from build123d import *

# Parameters (mm, degrees)
SKETCH1_R           = 2.9
BOSS_EXTRUDE1_DEPTH = 6.35
BOSS_EXTRUDE2_START = -6.35
SKETCH2_R           = 2.9
SKETCH2_R_2         = 2.6035
BOSS_EXTRUDE2_DEPTH = 6.35


with BuildPart() as part:
    # Sketch1 → Boss-Extrude1 (new body)
    with BuildSketch(Plane(origin=(0, 0, 0), x_dir=(1, 0, 0), z_dir=(0, 1, 0))):
        with BuildLine():
            Line((0, 5.08), (50.8, 5.08))
            ThreePointArc((50.8, 5.08), (55.88, 0), (50.8, -5.08))
            Line((50.8, -5.08), (0, -5.08))
            ThreePointArc((0, -5.08), (-5.08, 0), (0, 5.08))
        make_face()
        with Locations(Location((0, 0, 0), (0, 0, 270))):
            Circle(SKETCH1_R, mode=Mode.SUBTRACT)
        with Locations(Location((50.8, 0, 0), (0, 0, 270))):
            Circle(SKETCH1_R, mode=Mode.SUBTRACT)
    extrude(amount=BOSS_EXTRUDE1_DEPTH)

    # Sketch2 → Boss-Extrude2 (add)
    # profile 1 of 2: a face of its own
    with BuildSketch(Plane(origin=(0, 6.35, 0), x_dir=(1, 0, 0), z_dir=(0, 1, 0)).offset(BOSS_EXTRUDE2_START)):
        Circle(SKETCH2_R)
        with Locations(Location((0, 0, 0), (0, 0, 270))):
            Circle(SKETCH2_R_2, mode=Mode.SUBTRACT)
    # profile 2 of 2: a face of its own
    with BuildSketch(Plane(origin=(0, 6.35, 0), x_dir=(1, 0, 0), z_dir=(0, 1, 0)).offset(BOSS_EXTRUDE2_START)):
        with Locations((50.8, 0)):
            Circle(SKETCH2_R)
        with Locations(Location((50.8, 0, 0), (0, 0, 270))):
            Circle(SKETCH2_R_2, mode=Mode.SUBTRACT)
    extrude(amount=BOSS_EXTRUDE2_DEPTH)


solid = part.part
The model under review builds one solid part; all positions refer to its coordinate system, in mm. Round coordinates to 2 decimals unless told otherwise and drop trailing zeros. Order: outer loops, then holes, each group sorted by start corner. A loop starts at its lowest first (then second) coordinate and runs counter-clockwise, first axis right, second up. Notation, with made-up numbers: (-21.5, 33) -> (36.5, 33) arc R32 ccw to (36.5, 62) -> close; hole circle Ø11 at (57.25, -36.75). An arc over 180 degrees is marked (long way). Return JSON: item names as keys, results as strings.
1. The part is to be moulded in two halves that separate along X. For faces 1 (the face through (0.782, 3.131, 2.483)), 2 (the face through (55.88, 3.13, -0.11)), 3 (the face through (-5.08, 3.13, 0.11)), 4 (the face through (25, 6.35, 0)), say which applies: +X half, -X half, draft (parallel to the pull), parting line (faces both ways), or undercut.
Answer block:
{"face 1": "undercut", "face 2": "+X half", "face 3": "-X half", "face 4": "draft"}
2. Take a section at C-C (y = 3.25). Write out the cut boundary in (x, z).
Answer block:
{"outline": "(0, -5.08) -> (50.8, -5.08) arc R5.08 ccw to (50.8, 5.08) -> (0, 5.08) arc R5.08 ccw to start; hole circle Ø5.21 at (0, 0); hole circle Ø5.21 at (50.8, 0)"}
3. Take a section at A-A (z = 0). Write out the cut boundary in (x, y).
Answer block:
{"outline": "(-5.08, 0) -> (-2.6, 0) -> (-2.6, 6.35) -> (-5.08, 6.35) -> close; (2.6, 0) -> (48.2, 0) -> (48.2, 6.35) -> (2.6, 6.35) -> close; (53.4, 0) -> (55.88, 0) -> (55.88, 6.35) -> (53.4, 6.35) -> close"}
4. Insertion check: P1, Ø4.5, axis at x = 50.8, z = 0, coming from the -Y side. The pin has a flat end and moves straight along its axis. Give the tip position at first contact, or say it passes through.
Answer block:
{"P1": "passes through"}
5. Take a section at B-B (x = -1). Write out the cut boundary in (y, z).
Answer block:
{"outline": "(0, -4.98) -> (6.35, -4.98) -> (6.35, -2.4) -> (0, -2.4) -> close; (0, 2.4) -> (6.35, 2.4) -> (6.35, 4.98) -> (0, 4.98) -> close"}
6. Take a section at D-D (z = 3.5). Write out the cut boundary in (x, y).
Answer block:
{"outline": "(-3.68, 0) -> (54.48, 0) -> (54.48, 6.35) -> (-3.68, 6.35) -> close"}
7. For L1, parallel to X at y = 5.25, z = 0; L2, parallel to X at y = 4, z = 2.25; L3, parallel to Z at x = 0.5, y = 1.75, list the stretches that pass through material, from the lowest coordinate up. Write a range as [from, to].
Answer block:
{"L1": "x = [-5.08, -2.6], [2.6, 48.2], [53.4, 55.88]", "L2": "x = [-4.55, -1.31], [1.31, 49.49], [52.11, 55.35]", "L3": "z = [-5.08, -2.56], [2.56, 5.08]"}
